```python
from build123d import *

# Parameters (mm, degrees)
BRACKET_BODY_DEPTH    = 40
ROUNDED_LUG_CUT_DEPTH = 80
PIN_HOLE_SKETCH_R     = 7.5
PIN_HOLE_15_DEPTH     = 80
FORK_GAP_SKETCH_R     = 6
FORK_GAP_12MM_DEPTH   = 80
ARM_SLOTS_2X6_5_DEPTH = 80


with BuildPart() as part:
    # Bracket Profile Sketch → Bracket Body (new, symmetric)
    with BuildSketch(Plane.XY):
        Polygon((0, 0), (58, 0), (58, 13), (17, 13), (17, 47), (58, 47), (58, 60), (17, 60), (17, 130), (0, 130), align=None)
    extrude(amount=BRACKET_BODY_DEPTH, both=True)

    # Lug Shape Sketch → Rounded Lug Cut (cut)
    with BuildSketch(Plane(origin=(17, 0, 0), x_dir=(0, 0, -1), z_dir=(1, 0, 0))):
        with BuildLine():
            Line((40, 130), (9.4e-08, 130))
            ThreePointArc((9.4e-08, 130), (22.043839272, 120.869142787), (31.174696418, 98.825303582))
            Line((31.174696418, 98.825303582), (31.174696418, 69.93076474))
            ThreePointArc((31.174696418, 69.93076474), (33.699839758, 63.287985359), (40, 60))
            Line((40, 60), (40, 130))
        make_face()
        with BuildLine():
            Line((-31.174696418, 69.93076474), (-31.174696418, 98.825303582))
            ThreePointArc((-31.174696418, 98.825303582), (-22.043839205, 120.869142854), (9.4e-08, 130))
            Line((9.4e-08, 130), (-40, 130))
            Line((-40, 130), (-40, 60))
            ThreePointArc((-40, 60), (-33.699839758, 63.287985359), (-31.174696418, 69.93076474))
        make_face()
    extrude(amount=-ROUNDED_LUG_CUT_DEPTH, mode=Mode.SUBTRACT)

    # Pin Hole Sketch → Pin Hole Ø15 (cut)
    with BuildSketch(Plane(origin=(17, 0, 0), x_dir=(0, 0, -1), z_dir=(1, 0, 0))):
        with Locations((0, 98.825303582)):
            Circle(PIN_HOLE_SKETCH_R)
    extrude(amount=-PIN_HOLE_15_DEPTH, mode=Mode.SUBTRACT)

    # Fork Gap Sketch → Fork Gap 12mm (cut)
    with BuildSketch(Plane(origin=(17, 0, 0), x_dir=(0, 0, -1), z_dir=(1, 0, 0))):
        with Locations((-21.5, 30)):
            Circle(FORK_GAP_SKETCH_R)
        with Locations((21.5, 30)):
            Circle(FORK_GAP_SKETCH_R)
    extrude(amount=-FORK_GAP_12MM_DEPTH, mode=Mode.SUBTRACT)

    # Arm Slots Sketch → Arm Slots 2x6.5 (cut)
    with BuildSketch(Plane(origin=(0, 60, 0), x_dir=(1, 0, 0), z_dir=(0, 1, 0))):
        with BuildLine():
            Line((38.5, -26), (38.5, 26))
            ThreePointArc((38.5, 26), (45, 32.5), (51.5, 26))
            Line((51.5, 26), (51.5, -26))
            ThreePointArc((51.5, -26), (45, -32.5), (38.5, -26))
        make_face()
    extrude(amount=-ARM_SLOTS_2X6_5_DEPTH, mode=Mode.SUBTRACT)


solid = part.part
```
Part model, mm, in its own coordinate system. A direction names the side the tool comes from. Round coordinates to 2 decimals unless told otherwise and drop trailing zeros. Order: outer loops, then holes, each group sorted by start corner. A loop starts at its lowest first (then second) coordinate and runs counter-clockwise, first axis right, second up. Notation, with made-up numbers: M 34.5,86.5 L 49.5,86.5 A11 cw 49.5,94.5 Z; hole C 35.5,68.25 d3. An arc over 180 degrees is marked long. Answer in a Markdown table with one row per item. Add a question column.
Q1. Cut at D-D on z = 23. Give the cut face in (x, y), and give its area (3 significant figures).
Q2. 3-axis set-ups, long thin cutter, end or side, ignore diameter. For faces 5 (the face through (51.5, 7, 0)), 6 (the face through (9, 84, 31.175)), 7 (the face through (17, 30, 1)): which of +Z, -Z, +X, -X, +Y, -Y reach the whole face in a straight line?
Q3. Cut at C-C on x = 45. Give the cut face in (y, z), and give its area (3 significant figures).
Q4. Mould opens along Z. For faces 1 (the face through (44.9, 6.6, -32.5)), 2 (the face through (33, 13, 1)), 3 (the face through (16, 30, -40)), 4 (the face through (8.619, 24.143, -20.199)) say: +Z half, -Z half, draft (parallel to the pull), parting line (faces both ways), or undercut.
Q5. Wall check: L1, parallel to X at y = 6, z = -1.5; L2, parallel to Y at x = 29, z = -4; L3, parallel to Y at x = 9, z = 0. Give the ranges that are in metal, low to high. Write a range as from..to.
Q6. Pin check, flat tips, straight feed: pin 1 (15.5 mm diameter, centred on y = 30, z = 21.5, fed in from +X); pin 2 (5 mm diameter, centred on x = 6, y = 82.5, fed in from +Z); pin 3 (20.5 mm diameter, centred on x = 44, z = 11.5, fed in from +Y). Stop position of each tip, or through.
Q7. Cut at B-B on x = 24. Give the cut face in (y, z).
Q8. Cut at A-A on y = 30. Give the cut face in (x, z), and give its area (3 significant figures).
Established:
| question | item | result |
|---|---|---|
| 1 | outline | M 0,0 L 38.5,0 L 38.5,13 L 17,13 L 17,24.19 L 0,24.19 Z; M 0,35.81 L 17,35.81 L 17,47 L 38.5,47 L 38.5,60 L 17,60 L 17,119.87 L 0,119.87 Z; M 51.5,0 L 58,0 L 58,13 L 51.5,13 Z; M 51.5,47 L 58,47 L 58,60 L 51.5,60 Z |
| 1 | area | 2,570 mm2 |
| 2 | face 5 | +Y, -Y |
| 2 | face 6 | +Z, +X, -X, +Y |
| 2 | face 7 | +Z, -Z, +X |
| 3 | outline | M 0,-40 L 13,-40 L 13,-32.5 L 0,-32.5 Z; M 0,32.5 L 13,32.5 L 13,40 L 0,40 Z; M 47,-40 L 60,-40 L 60,-32.5 L 47,-32.5 Z; M 47,32.5 L 60,32.5 L 60,40 L 47,40 Z |
| 3 | area | 390 mm2 |
| 4 | face 1 | undercut |
| 4 | face 2 | draft |
| 4 | face 3 | -Z half |
| 4 | face 4 | undercut |
| 5 | L1 | x = 0..38.5, 51.5..58 |
| 5 | L2 | y = 0..13, 47..60 |
| 5 | L3 | y = 0..91.33, 106.33..130 |
| 6 | pin 1 | stops at x = 17 |
| 6 | pin 2 | stops at z = 31.17 |
| 6 | pin 3 | stops at y = 60 |
| 7 | outline | M 0,-40 L 13,-40 L 13,40 L 0,40 Z; M 47,-40 L 60,-40 L 60,40 L 47,40 Z |
| 8 | outline | M 0,-40 L 17,-40 L 17,-27.5 L 0,-27.5 Z; M 0,-15.5 L 17,-15.5 L 17,15.5 L 0,15.5 Z; M 0,27.5 L 17,27.5 L 17,40 L 0,40 Z |
| 8 | area | 952 mm2 |
